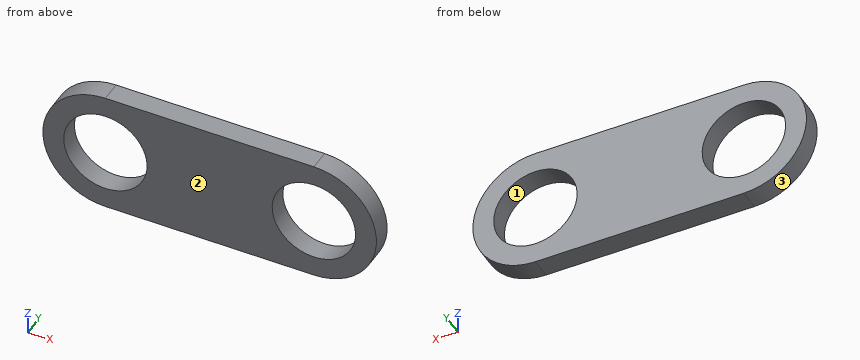
from build123d import *

# Parameters (mm, degrees)
SKETCH_1_R      = 20
EXTRUDE_1_DEPTH = 10


with BuildPart() as part:
    # 草图1 → 凸台-拉伸1 (new body)
    with BuildSketch(Plane(origin=(0, 0, 0), x_dir=(1, 0, 0), z_dir=(0, 1, 0))):
        with BuildLine():
            Line((-50, 30), (50, 30))
            ThreePointArc((50, 30), (80, 0), (50, -30))
            Line((50, -30), (-50, -30))
            ThreePointArc((-50, -30), (-80, 0), (-50, 30))
        make_face()
        with Locations(Location((50, 0, 0), (0, 0, 270))):
            Circle(SKETCH_1_R, mode=Mode.SUBTRACT)
        with Locations(Location((-50, 0, 0), (0, 0, 270))):
            Circle(SKETCH_1_R, mode=Mode.SUBTRACT)
    extrude(amount=EXTRUDE_1_DEPTH)


solid = part.part
Geometry check sheet. Reference: the model listing, model coordinates, mm. Face numbers are marked on the shaded views. Give positions to 0.01 mm unless a question says otherwise; leave off trailing zeros. Write each loop counter-clockwise with the first axis right and the second up, starting at its lowest first coordinate (ties: lowest second). Pieces come first, ordered by that corner, then holes.
1) Cross-section at A-A (z = 0). Record the boundary of the cut face in (x, y), plus the area to 3 significant figures.
Values follow:
outline: (-80, 0) - (-70, 0) - (-70, 10) - (-80, 10) - close; (-30, 0) - (30, 0) - (30, 10) - (-30, 10) - close; (70, 0) - (80, 0) - (80, 10) - (70, 10) - close
area: 800 mm2
2) Release check for a two-part mould opening along X. For the marked faces 1, 2 and 3 record: released by +X, released by -X, zero draft, split by the parting line, or undercut.
Values follow:
face 1: undercut
face 2: zero draft
face 3: released by -X
3) Thickness scan on line 1 (X direction, y = 2.5, z = 0); line 2 (X direction, y = 9.5, z = 4); line 3 (Z direction, x = -37.5, y = 9.25). Record the ranges inside material, lowest first.
Values follow:
line 1: x = -80 to -70, -30 to 30, 70 to 80
line 2: x = -79.73 to -69.6, -30.4 to 30.4, 69.6 to 79.73
line 3: z = -30 to -15.61, 15.61 to 30
4) Cross-section at B-B (x = -65.5). Record the boundary of the cut face in (y, z), plus the area to 3 significant figures.
Values follow:
outline: (0, -25.69) - (10, -25.69) - (10, -12.64) - (0, -12.64) - close; (0, 12.64) - (10, 12.64) - (10, 25.69) - (0, 25.69) - close
area: 261 mm2
5) Cross-section at C-C (y = 2.25). Record the boundary of the cut face in (x, z), plus the area to 3 significant figures.
Values follow:
outline: (-50, -30) - (50, -30) arc R30 ccw to (50, 30) - (-50, 30) arc R30 ccw to start; hole circle Ø40 at (-50, 0); hole circle Ø40 at (50, 0)
area: 6,310 mm2
6) Go/stop test with flat-tipped pins: pin 1 Ø2 at (y, z) = (5, 1.5) entering from +X; pin 2 Ø24 at (x, z) = (-50, 0) entering from -Y; pin 3 Ø6 at (y, z) = (4.5, -16) entering from +X; pin 4 Ø12 at (x, z) = (-30, -1) entering from -Y. Record where each tip stops, or that it passes through.
Values follow:
pin 1: stops at x = 80
pin 2: passes through
pin 3: stops at x = 77.04
pin 4: stops at y = 0
7) Cross-section at D-D (z = -9). Record the boundary of the cut face in (x, y), plus the area to 3 significant figures.
Values follow:
outline: (-78.62, 0) - (-67.86, 0) - (-67.86, 10) - (-78.62, 10) - close; (-32.14, 0) - (32.14, 0) - (32.14, 10) - (-32.14, 10) - close; (67.86, 0) - (78.62, 0) - (78.62, 10) - (67.86, 10) - close
area: 858 mm2
